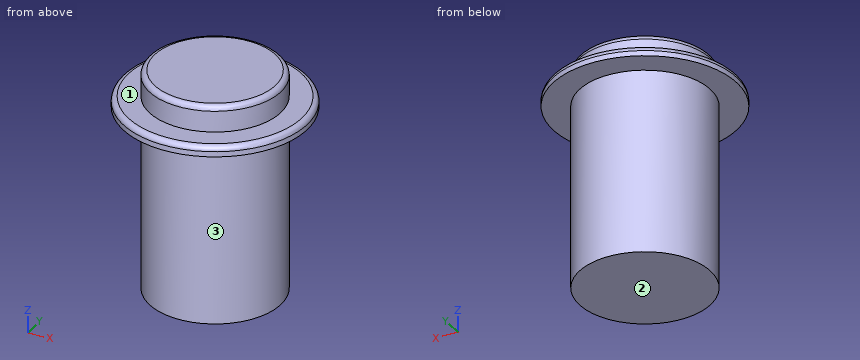
```python
from build123d import *

# Parameters (mm, degrees)
SKETCH1_R           = 12.5
BOSS_EXTRUDE1_DEPTH = 35
SKETCH2_R           = 17.5
BOSS_EXTRUDE2_DEPTH = 2
BOSS_EXTRUDE3_START = 5
SKETCH3_R           = 12.5
BOSS_EXTRUDE3_DEPTH = 5
FILLET1_R           = 1


with BuildPart() as part:
    # Sketch1 → Boss-Extrude1 (new body)
    with BuildSketch(Plane.XY):
        with Locations((336.110854844, 94.216541461)):
            Circle(SKETCH1_R)
    extrude(amount=-BOSS_EXTRUDE1_DEPTH)

    # Sketch2 → Boss-Extrude2 (add)
    with BuildSketch(Plane.XY):
        with Locations((336.110854844, 94.216541461)):
            Circle(SKETCH2_R)
    extrude(amount=BOSS_EXTRUDE2_DEPTH)

    # Sketch3 → Boss-Extrude3 (add)
    with BuildSketch(Plane.XY.offset(2).offset(BOSS_EXTRUDE3_START)):
        with Locations((336.110854844, 94.216541461)):
            Circle(SKETCH3_R)
    extrude(amount=-BOSS_EXTRUDE3_DEPTH)

    # Fillet1
    fillet1_edges = [part.edges().sort_by_distance(p)[0] for p in [
        (323.610854844, 94.216541461, 7),
        (318.610854844, 94.216541461, 2),
    ]]
    fillet(fillet1_edges, radius=FILLET1_R)


solid = part.part
```
The listing builds one solid part. Answer for the finished solid, in the listing's coordinates (mm). Face numbers are marked on the shaded views. A direction names the side the tool comes from. Give positions to 0.01 mm unless a question says otherwise; leave off trailing zeros. Loops run counter-clockwise (first coordinate to the right, second up) from the corner with the lowest first, then second, coordinate; pieces in that order, holes last. Notation, with made-up numbers: M 7.5,-5 L 60.5,-5 A22 cw 60.5,19 Z; hole C -19,44.5 d6. An arc over 180 degrees is marked long. One line per item, written item: value.
Q1. A cutting plane is placed at A-A on z = -19. Determine the outline of the cut face in (x, y), then the cut area to 3 significant figures.
Working result:
outline: C 336.11,94.22 d25
area: 491 mm^2
Q2. Flat-ended cylindrical pins translate along their axes: P1, Ø5, axis at y = 103, z = -19, coming from the +X side; P2, Ø1.5, axis at y = 104.5, z = -12, coming from the -X side; P3, Ø12, axis at y = 97, z = -22.5, coming from the +X side. Find the tip coordinate at first contact, or state that the pin passes through.
Working result:
P1: stops at x = 346.92
P2: stops at x = 328.03
P3: stops at x = 348.61
Q3. For the marked faces 1, 2 and 3, determine the directions among +Z, -Z, +X, -X, +Y, -Y from which every point of the face is accessible in a straight line to the end or side of a thin tool.
Working result:
face 1: +Z
face 2: -Z, +X, -X, +Y, -Y
face 3: -Z
Q4. Find the intervals of material crossed by line 1 (Z direction, x = 351, y = 101.5); line 2 (Y direction, x = 340, z = 4); line 3 (Y direction, x = 334, z = -5), in increasing order. Write a range as from..to.
Working result:
line 1: z = 0..2
line 2: y = 82.34..106.1
line 3: y = 81.9..106.54
